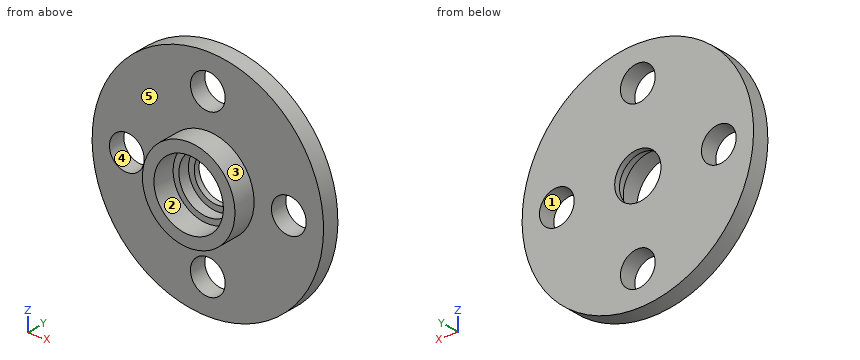
```python
from build123d import *

# Parameters (mm, degrees)
SKETCH2_R          = 1.5
CUT_EXTRUDE1_DEPTH = 10


with BuildPart() as part:
    # Sketch1 → Revolve1 (revolve)
    with BuildSketch(Plane.XY, mode=Mode.PRIVATE) as revolve1_sk:
        Polygon((-0.138513514, 1.280405405), (7.861486486, 1.280405405), (7.861486486, -0.219594595), (1.861486486, -0.219594595), (1.861486486, -1.019594595), (1.861486486, -2.219594595), (0.861486486, -2.219594595), (0.861486486, -0.219594595), (0.361486486, -0.219594595), (0.361486486, 0.780405405), (-0.138513514, 0.780405405), align=None)
    revolve(revolve1_sk.sketch.rotate(Axis((-2.138513514, 1.540540541, 0), (0, -1, 0)), 90), axis=Axis((-2.138513514, 1.540540541, 0), (0, -1, 0)))

    # Sketch2 → Cut-Extrude1 (cut)
    with BuildSketch(Plane(origin=(0, 1.280405405, 0), x_dir=(1, 0, 0), z_dir=(0, 1, 0))):
        with Locations(Location((-2.138513514, 7, 0), (0, 0, 270))):
            Circle(SKETCH2_R)
        with Locations(Location((4.861486486, 0, 0), (0, 0, 270))):
            Circle(SKETCH2_R)
        with Locations(Location((-2.138513514, -7, 0), (0, 0, 269.999999999))):
            Circle(SKETCH2_R)
        with Locations(Location((-9.138513514, 0, 0), (0, 0, 270))):
            Circle(SKETCH2_R)
    extrude(amount=-CUT_EXTRUDE1_DEPTH, mode=Mode.SUBTRACT)


solid = part.part
```
CAD build for the part. Positions are in the model's coordinates, mm. Face numbers are marked on the shaded views. A direction names the side the tool comes from. Coordinates: 2 decimals unless noted, no trailing zeros. Write each loop counter-clockwise with the first axis right and the second up, starting at its lowest first coordinate (ties: lowest second). Pieces come first, ordered by that corner, then holes. Notation, with made-up numbers: (15, -17.75) -> (56, -17.75) arc R29 ccw to (56, 11.25) -> close; hole circle Ø10 at (43, 53). An arc over 180 degrees is marked (long way). Use CSV: the item, a comma, the result in double quotes. Start each with the question number.
Item 1: Drop flat-ended pins along their axis: P1, Ø4.5, axis at x = -2.14, z = 0, coming from the -Y side; P2, Ø4, axis at x = -2.5, z = -0.5, coming from the -Y side; P3, Ø1.8, axis at x = -2.14, z = 7, coming from the -Y side; P4, Ø1, axis at x = 5.5, y = 0.5, coming from the +Z side. Give the stop position or say it passes through.
Item 2: Wall check: probe 1 along X at (y, z) = (0.25, 0); probe 2 along X at (y, z) = (1.05, 0); probe 3 along Z at (x, y) = (-2, -1.3). Give the ranges that are in metal, low to high.
Item 3: Band-saw the part on D-D, the plane y = 0.1. Write the cut outline in (x, z).
Item 4: Tool access for the marked faces 1 and 2: list every direction of +Z, -Z, +X, -X, +Y, -Y with a clear straight run to the whole face (end or side of a thin tool).
Item 5: Band-saw the part on A-A, the plane z = 0. Write the cut outline in (x, y), plus the area to 3 significant figures.
Item 6: Band-saw the part on C-C, the plane z = 7. Write the cut outline in (x, y), plus the area to 3 significant figures.
Item 7: Two-plate mould, pull along X, no slides. Class the marked faces 3, 4 and 5: +X half, -X half, draft (parallel to the pull), parting line (faces both ways), or undercut.
Item 8: Band-saw the part on B-B, the plane x = -8.75. Write the cut outline in (y, z), plus the area to 3 significant figures.
Response values:
1,P1,"stops at y = 0.78"
1,P2,"stops at y = -0.22"
1,P3,"passes through"
1,P4,"stops at z = 7"
2,probe 1,"x = -12.14 to -10.64, -7.64 to -4.64, 0.36 to 3.36, 6.36 to 7.86"
2,probe 2,"x = -12.14 to -10.64, -7.64 to -4.14, -0.14 to 3.36, 6.36 to 7.86"
2,probe 3,"z = -4 to -3, 3 to 4"
3,outline,"circle Ø20 at (-2.14, 0); hole circle Ø3 at (-9.14, 0); hole circle Ø5 at (-2.14, 0); hole circle Ø3 at (-2.14, -7); hole circle Ø3 at (-2.14, 7); hole circle Ø3 at (4.86, 0)"
4,face 1,"+Y, -Y"
4,face 2,"-Y"
5,outline,"(-12.14, -0.22) -> (-10.64, -0.22) -> (-10.64, 1.28) -> (-12.14, 1.28) -> close; (-7.64, -0.22) -> (-6.14, -0.22) -> (-6.14, -2.22) -> (-5.14, -2.22) -> (-5.14, -0.22) -> (-4.64, -0.22) -> (-4.64, 0.78) -> (-4.14, 0.78) -> (-4.14, 1.28) -> (-7.64, 1.28) -> close; (-0.14, 0.78) -> (0.36, 0.78) -> (0.36, -0.22) -> (0.86, -0.22) -> (0.86, -2.22) -> (1.86, -2.22) -> (1.86, -0.22) -> (3.36, -0.22) -> (3.36, 1.28) -> (-0.14, 1.28) -> close; (6.36, -0.22) -> (7.86, -0.22) -> (7.86, 1.28) -> (6.36, 1.28) -> close"
5,area,"18.0 mm2"
6,outline,"(-9.28, -0.22) -> (-3.64, -0.22) -> (-3.64, 1.28) -> (-9.28, 1.28) -> close; (-0.64, -0.22) -> (5, -0.22) -> (5, 1.28) -> (-0.64, 1.28) -> close"
6,area,"16.9 mm2"
7,face 3,"parting line"
7,face 4,"undercut"
7,face 5,"draft"
8,outline,"(-0.22, -7.5) -> (1.28, -7.5) -> (1.28, -1.45) -> (-0.22, -1.45) -> close; (-0.22, 1.45) -> (1.28, 1.45) -> (1.28, 7.5) -> (-0.22, 7.5) -> close"
8,area,"18.2 mm2"
